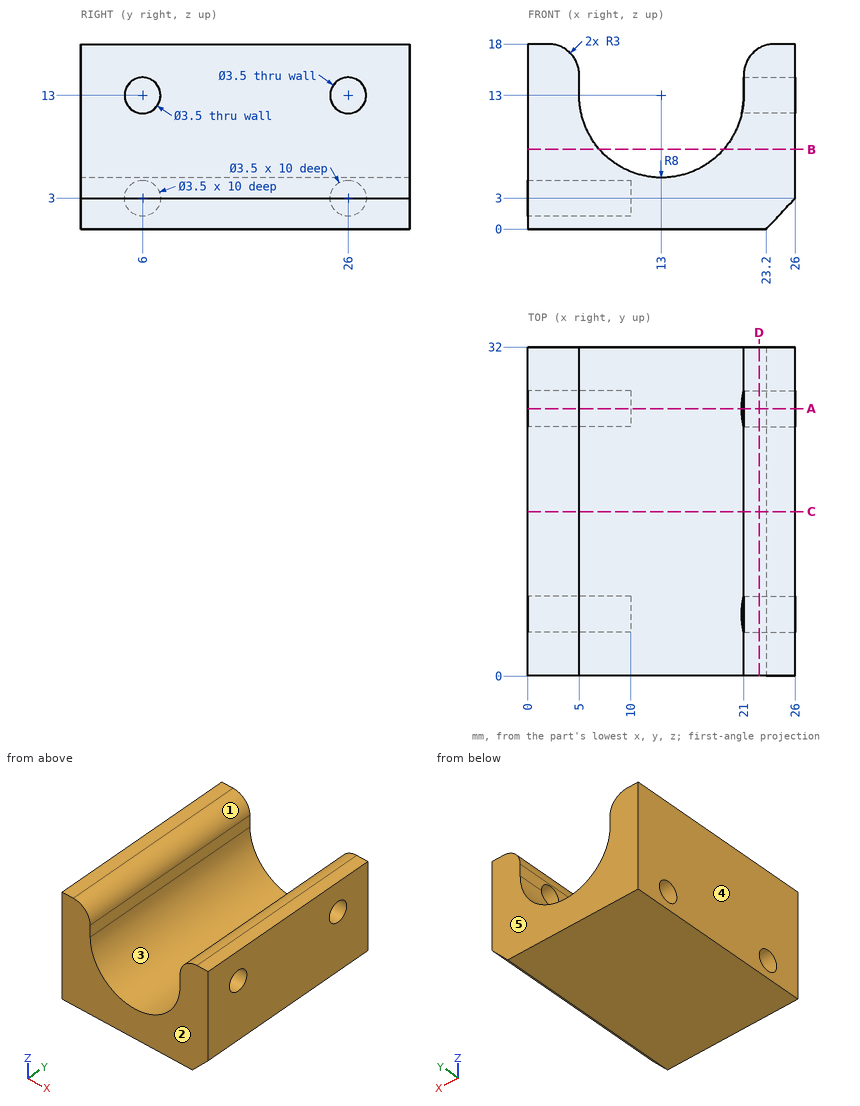
For this review, use the dimensioned drawing (mm, ordinates from the lowest corner) and the shaded views. A direction names the side the tool comes from. Round coordinates to 2 decimals unless told otherwise and drop trailing zeros. Loops run counter-clockwise (first coordinate to the right, second up) from the corner with the lowest first, then second, coordinate; pieces in that order, holes last. Notation, with made-up numbers: M 15.5,9 L 37.5,9 A30 cw 37.5,42 Z; hole C 24.25,-5 d1. An arc over 180 degrees is marked long. Answer as a JSON object with one key per item and string values.
(1) Clearance check with flat-ended pins moving along their axes: P1, Ø3, axis at x = 15, y = 13.5, coming from the +Z side; P2, Ø1, axis at y = 6, z = 3, coming from the -X side; P3, Ø1, axis at x = 4.5, y = 16, coming from the +Z side. State where each tip first meets the part, or that it passes through.
Resolved:
{"P1": "z = 5.81", "P2": "x = 10", "P3": "z = 17.24"}
(2) Take a section at A-A on y = 26. Give the boundary of the cut face in (x, z).
Resolved:
{"outline": "M 0,0 L 23.2,0 L 26,3 L 26,11.25 L 20.81,11.25 A8 cw 5,13 L 5,15 A3 ccw 2,18 L 0,18 L 0,4.75 L 10,4.75 L 10,1.25 L 0,1.25 Z; M 21,14.75 L 26,14.75 L 26,18 L 24,18 A3 ccw 21,15 Z"}
(3) Tool access review of the marked faces 1 and 2: name each direction out of +Z, -Z, +X, -X, +Y, -Y from which nothing blocks a thin tool from reaching the whole face with its end or side.
Resolved:
{"face 1": "+Z, +Y, -Y", "face 2": "+Z, -Z, +X, -X, -Y"}
(4) Take a section at D-D on x = 22.5. Give the boundary of the cut face in (y, z).
Resolved:
{"outline": "M 0,0 L 32,0 L 32,17.6 L 0,17.6 Z; hole C 6,13 d3.5; hole C 26,13 d3.5"}
(5) Draft analysis for pull direction X (two halves, no side actions). For the marked faces 3, 4 and 5, state which applies: released by +X, released by -X, zero draft, split by the parting line, or undercut.
Resolved:
{"face 3": "undercut", "face 4": "released by -X", "face 5": "zero draft"}
(6) To check wall thickness, follow line 1 along Y through (x, z) = (23.05, 13); line 2 along X through (y, z) = (19, 14.25); line 3 along Y through (x, z) = (3, 4.25). State the ranges of each line that lie inside material, in increasing order.
Resolved:
{"line 1": "0 to 4.25, 7.75 to 24.25, 27.75 to 32", "line 2": "0 to 5, 21 to 26", "line 3": "0 to 4.78, 7.22 to 24.78, 27.22 to 32"}
(7) Take a section at B-B on z = 7.75. Give the boundary of the cut face in (x, y).
Resolved:
{"outline": "M 0,0 L 6.96,0 L 6.96,32 L 0,32 Z; M 19.04,0 L 26,0 L 26,32 L 19.04,32 Z"}
(8) Take a section at C-C on y = 16. Give the boundary of the cut face in (x, z).
Resolved:
{"outline": "M 0,0 L 23.2,0 L 26,3 L 26,18 L 24,18 A3 ccw 21,15 L 21,13 A8 cw 5,13 L 5,15 A3 ccw 2,18 L 0,18 Z"}
